```python
from build123d import *

# Parameters (mm, degrees)
FLANGE_PLATE_SKETCH_R     = 5
FLANGE_PLATE_DEPTH        = 10
FLANGE_START              = -5
FLANGE_RECESS_SKETCH_R    = 7.5
FLANGE_RECESS_SKETCH_R_2  = 5
FLANGE_RECESS_5MM_DEPTH   = 5
BRACKET_BODY_SKETCH_R     = 2.5
BRACKET_BODY_DEPTH        = 50
THROUGH_START             = -50
THROUGH_BORE_SKETCH_R     = 10
THROUGH_BORE_DEPTH        = 50
BORE_COUNTERBORE_SKETCH_R = 12
BORE_COUNTERBORE_24_DEPTH = 5
BODY_POCKET_SKETCH_R      = 5
BODY_POCKET_20MM_DEPTH    = 20
POCKET_STEP_SKETCH_R      = 7.5
POCKET_STEP_3MM_DEPTH     = 3
BODY_BOSS_12MM_DEPTH      = 12
BODY_FILLET_R8_A_R        = 8
BODY_FILLET_R8_B_R        = 8
BODY_SLOT_SKETCH_R        = 2.5
BODY_SLOT_CUT_DEPTH       = 112.126054551


with BuildPart() as part:
    # Flange Plate Sketch → Flange Plate (new body)
    with BuildSketch(Plane.XY):
        with BuildLine():
            Line((-35, -46), (-35, 14))
            ThreePointArc((-35, 14), (0, 49), (35, 14))
            Line((35, 14), (35, -46))
            ThreePointArc((35, -46), (0, -81), (-35, -46))
        make_face()
        with Locations((-25, 0)):
            Circle(FLANGE_PLATE_SKETCH_R, mode=Mode.SUBTRACT)
        with Locations((25, 0)):
            Circle(FLANGE_PLATE_SKETCH_R, mode=Mode.SUBTRACT)
        with Locations((-25, -32)):
            Circle(FLANGE_PLATE_SKETCH_R, mode=Mode.SUBTRACT)
        with Locations((25, -32)):
            Circle(FLANGE_PLATE_SKETCH_R, mode=Mode.SUBTRACT)
    extrude(amount=FLANGE_PLATE_DEPTH)

    # Flange Recess Sketch → Flange Recess 5mm (cut)
    # profile 1 of 4: a face of its own
    with BuildSketch(Plane.XY.offset(10).offset(FLANGE_START)):
        with Locations((-25, 0)):
            Circle(FLANGE_RECESS_SKETCH_R)
        with Locations((-25, 0)):
            Circle(FLANGE_RECESS_SKETCH_R_2, mode=Mode.SUBTRACT)
    # profile 2 of 4: a face of its own
    with BuildSketch(Plane.XY.offset(10).offset(FLANGE_START)):
        with Locations((25, 0)):
            Circle(FLANGE_RECESS_SKETCH_R)
        with Locations((25, 0)):
            Circle(FLANGE_RECESS_SKETCH_R_2, mode=Mode.SUBTRACT)
    # profile 3 of 4: a face of its own
    with BuildSketch(Plane.XY.offset(10).offset(FLANGE_START)):
        with Locations((25, -32)):
            Circle(FLANGE_RECESS_SKETCH_R)
        with Locations((25, -32)):
            Circle(FLANGE_RECESS_SKETCH_R_2, mode=Mode.SUBTRACT)
    # profile 4 of 4: a face of its own
    with BuildSketch(Plane.XY.offset(10).offset(FLANGE_START)):
        with Locations((-25, -32)):
            Circle(FLANGE_RECESS_SKETCH_R)
        with Locations((-25, -32)):
            Circle(FLANGE_RECESS_SKETCH_R_2, mode=Mode.SUBTRACT)
    extrude(amount=FLANGE_RECESS_5MM_DEPTH, mode=Mode.SUBTRACT)

    # Bracket Body Sketch → Bracket Body (add)
    # profile 1 of 2: a face of its own
    with BuildSketch(Plane.XY.offset(10)):
        with BuildLine():
            Line((-12.5, -72), (-23.430749028, -72))
            ThreePointArc((-23.430749028, -72), (0, -81), (23.430749028, -72))
            Line((23.430749028, -72), (12.5, -72))
            ThreePointArc((12.5, -72), (7.458524391, -70.211563707), (4.67113827, -65.645880922))
            ThreePointArc((4.67113827, -65.645880922), (4.822624016, -64.374561693), (5.714098019, -63.455608694))
            ThreePointArc((5.714098019, -63.455608694), (10.669494488, -58.85053718), (12.5, -52.33809621))
            Line((12.5, -52.33809621), (12.5, -9.987492178))
            ThreePointArc((12.5, -9.987492178), (15.954701786, -1.203117164), (13.856406461, 8))
            Line((13.856406461, 8), (7.473378872, 19.05572809))
            ThreePointArc((7.473378872, 19.05572809), (0, 24.201151372), (-7.473378872, 19.05572809))
            Line((-7.473378872, 19.05572809), (-13.856406461, 8))
            ThreePointArc((-13.856406461, 8), (-15.954701786, -1.203117164), (-12.5, -9.987492178))
            Line((-12.5, -9.987492178), (-12.5, -52.33809621))
            ThreePointArc((-12.5, -52.33809621), (-10.669494488, -58.85053718), (-5.714098019, -63.455608694))
            ThreePointArc((-5.714098019, -63.455608694), (-4.822624016, -64.374561693), (-4.67113827, -65.645880922))
            ThreePointArc((-4.67113827, -65.645880922), (-7.458524391, -70.211563707), (-12.5, -72))
        make_face()
        with Locations((0, -20)):
            Circle(BRACKET_BODY_SKETCH_R, mode=Mode.SUBTRACT)
        with BuildLine():
            ThreePointArc((0, -10), (-7.071067812, 7.071067812), (10, 0))
            ThreePointArc((10, 0), (7.071067812, -7.071067812), (0, -10))
        make_face(mode=Mode.SUBTRACT)
        with Locations((0, 16)):
            Circle(BRACKET_BODY_SKETCH_R, mode=Mode.SUBTRACT)
    # profile 2 of 2: a face of its own
    with BuildSketch(Plane.XY.offset(10)):
        with BuildLine():
            Line((-45, -72), (-45, -82))
            Line((-45, -82), (45, -82))
            Line((45, -82), (45, -72))
            Line((45, -72), (23.430749028, -72))
            ThreePointArc((23.430749028, -72), (0, -81), (-23.430749028, -72))
            Line((-23.430749028, -72), (-45, -72))
        make_face()
    extrude(amount=BRACKET_BODY_DEPTH)

    # Through Bore Sketch → Through Bore (cut)
    with BuildSketch(Plane.XY.offset(10).offset(THROUGH_START)):
        with Locations(Location((0, 0, 0), (0, 0, 180))):
            Circle(THROUGH_BORE_SKETCH_R)
    extrude(amount=THROUGH_BORE_DEPTH, mode=Mode.SUBTRACT)

    # Bore Counterbore Sketch → Bore Counterbore Ø24 (cut)
    with BuildSketch(Plane.XY.offset(60)):
        Circle(BORE_COUNTERBORE_SKETCH_R)
    extrude(amount=-BORE_COUNTERBORE_24_DEPTH, mode=Mode.SUBTRACT)

    # Body Pocket Sketch → Body Pocket 20mm (cut)
    with BuildSketch(Plane(origin=(0, -72, 0), x_dir=(1, 0, 0), z_dir=(0, 1, 0))):
        with Locations(Location((-31.350256263, -20, 0), (0, 0, 270))):
            Circle(BODY_POCKET_SKETCH_R)
        with Locations(Location((-31.350256263, -50, 0), (0, 0, 270))):
            Circle(BODY_POCKET_SKETCH_R)
        with Locations(Location((33.649743737, -20, 0), (0, 0, 270))):
            Circle(BODY_POCKET_SKETCH_R)
        with Locations(Location((33.649743737, -50, 0), (0, 0, 270))):
            Circle(BODY_POCKET_SKETCH_R)
    extrude(amount=-BODY_POCKET_20MM_DEPTH, mode=Mode.SUBTRACT)

    # Pocket Step Sketch → Pocket Step 3mm (cut)
    with BuildSketch(Plane(origin=(0, -72, 0), x_dir=(1, 0, 0), z_dir=(0, 1, 0))):
        with Locations(Location((-31.350256263, -20, 0), (0, 0, 270))):
            Circle(POCKET_STEP_SKETCH_R)
        with Locations(Location((-31.350256263, -50, 0), (0, 0, 270))):
            Circle(POCKET_STEP_SKETCH_R)
        with Locations(Location((33.649743737, -20, 0), (0, 0, 270))):
            Circle(POCKET_STEP_SKETCH_R)
        with Locations(Location((33.649743737, -50, 0), (0, 0, 270))):
            Circle(POCKET_STEP_SKETCH_R)
    extrude(amount=-POCKET_STEP_3MM_DEPTH, mode=Mode.SUBTRACT)

    # Body Boss Sketch → Body Boss 12mm (add)
    with BuildSketch(Plane.XY.offset(10)):
        with BuildLine():
            Line((7.473378872, 19.05572809), (5.820364134, 25.658327183))
            ThreePointArc((5.820364134, 25.658327183), (0, 30.201151372), (-5.820364134, 25.658327183))
            Line((-5.820364134, 25.658327183), (-7.473378872, 19.05572809))
            ThreePointArc((-7.473378872, 19.05572809), (0, 24.201151372), (7.473378872, 19.05572809))
        make_face()
    extrude(amount=BODY_BOSS_12MM_DEPTH)

    # Body Fillet R8 A
    body_fillet_r8_a_edges = [part.edges().sort_by_distance(p)[0] for p in [
        (-45, -77, 60),
        (45, -77, 60),
    ]]
    fillet(body_fillet_r8_a_edges, radius=BODY_FILLET_R8_A_R)

    # Body Fillet R8 B
    body_fillet_r8_b_edges = [part.edges().sort_by_distance(p)[0] for p in [
        (-45, -77, 10),
        (45, -77, 10),
    ]]
    fillet(body_fillet_r8_b_edges, radius=BODY_FILLET_R8_B_R)

    # Body Slot Sketch → Body Slot Cut (cut, through all)
    with BuildSketch(Plane.XY.offset(60)):
        with Locations((0, 16)):
            Circle(BODY_SLOT_SKETCH_R)
        with Locations((0, -20)):
            Circle(BODY_SLOT_SKETCH_R)
    extrude(amount=-BODY_SLOT_CUT_DEPTH, mode=Mode.SUBTRACT)


solid = part.part
```
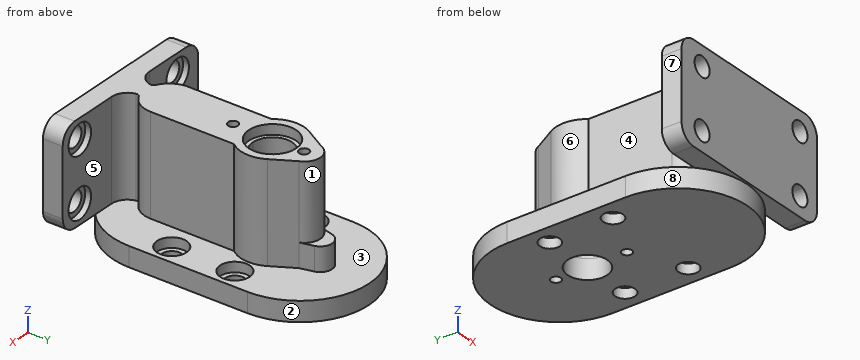
Model file for the job. Use its own axes, mm. Face numbers are marked on the shaded views. A direction names the side the tool comes from. Coordinates: 2 decimals unless noted, no trailing zeros. Loops run counter-clockwise (first coordinate to the right, second up) from the corner with the lowest first, then second, coordinate; pieces in that order, holes last. Notation, with made-up numbers: (-33, 39) - (12, 39) arc R24 ccw to (12, 77) - close; hole circle Ø3 at (42, 28.5). An arc over 180 degrees is marked (long way). Answer as a JSON object with one key per item and string values. Group by question number.
(1) Tool access for the marked faces 1, 2, 3, 4 and 5: list every direction of +Z, -Z, +X, -X, +Y, -Y with a clear straight run to the whole face (end or side of a thin tool).
(2) Probe line 1 along Y through (x, z) = (7, 35); line 2 along Y through (x, z) = (-25, 1); line 3 along X through (y, z) = (-80, 50). List the from-to ranges inside material, lowest first.
(3) Two-plate mould, pull along Y, no slides. Class the marked faces 6, 7 and 8: released by +Y, released by -Y, zero draft, split by the parting line, or undercut.
(4) Flat gauge pins, fed straight in: pin 1 (6 mm diameter, centred on y = -53.5, z = 20, fed in from -X); pin 2 (9 mm diameter, centred on x = 25, y = -32, fed in from +Z); pin 3 (7.5 mm diameter, centred on x = 35, z = 23, fed in from +Y); pin 4 (3 mm diameter, centred on y = -3.5, z = 4, fed in from -X). Where does each tip first touch, or does it go through?
(5) Cut at A-A (z = 32). Give the cut face in (x, y).
(6) Cut at C-C (z = 50). State how many separate pieces and enclosed holes the cut face has, then the cut area to 3 significant figures.
(7) Cut at B-B (y = -20). Give the cut face in (x, z).
Geometry says:
{
 "1": {"face 1": "+Z, +Y", "face 2": "+Z, -Z, +Y", "face 3": "+Z", "face 4": "+Z, -X", "face 5": "+Z, +X"},
 "2": {"line 1": "y = -82 to -69.81, -62.69 to -7.14, 7.14 to 20.07", "line 2": "y = -70.49 to -37, -27 to -5, 5 to 38.49", "line 3": "x = -45 to -36.35, -26.35 to 28.65, 38.65 to 45"},
 "3": {"face 6": "undercut", "face 7": "zero draft", "face 8": "released by -Y"},
 "4": {"pin 1": "stops at x = -12.5", "pin 2": "passes through", "pin 3": "stops at y = -75", "pin 4": "stops at x = -35"},
 "5": {"outline": "(-45, -82) - (45, -82) - (45, -72) - (12.5, -72) arc R8 cw to (4.67, -65.65) arc R2 cw to (5.71, -63.46) arc R12.5 ccw to (12.5, -52.34) - (12.5, -9.99) arc R16 ccw to (13.86, 8) - (7.47, 19.06) arc R8 ccw to (-7.47, 19.06) - (-13.86, 8) arc R16 ccw to (-12.5, -9.99) - (-12.5, -52.34) arc R12.5 ccw to (-5.71, -63.46) arc R2 cw to (-4.67, -65.65) arc R8 cw to (-12.5, -72) - (-45, -72) - close; hole circle Ø20 at (0, 0); hole circle Ø5 at (0, -20); hole circle Ø5 at (0, 16)"},
 "6": {"separate pieces": "3", "enclosed holes": "3", "area": "2,550 mm^2"},
 "7": {"outline": "(-35, 0) - (-2.5, 0) - (-2.5, 60) - (-12.5, 60) - (-12.5, 10) - (-35, 10) - close; (2.5, 0) - (35, 0) - (35, 10) - (12.5, 10) - (12.5, 60) - (2.5, 60) - close"}
}
